Read the model definition and answer for the solid it produces. Units are mm, in the model's axes. A direction names the side the tool comes from. Give positions to 0.01 mm unless a question says otherwise; leave off trailing zeros. Loops run counter-clockwise (first coordinate to the right, second up) from the corner with the lowest first, then second, coordinate; pieces in that order, holes last.
(1) Find section B-B, the plane y = 0. Write down the section's boundary in (x, z), then the cut area to 3 significant figures.
(2) Determine the mould class of faces 6 (the face through (112, 7, 16)), 7 (the face through (7.048, 7.583, -12.942)), 8 (the face through (63.674, -12.447, -2.764)) for opening direction Z: pulls with the +Z half, pulls with the -Z half, needs draft (parallel to the pull), parting line crosses it, or undercut.
(3) Find section A-A, the plane z = 0. Write down the section's boundary in (x, y), then the cut area to 3 significant figures.
(4) Straight lines are drawn through the part: probe 1 along Y at (x, z) = (76, 0); probe 2 along Y at (x, z) = (72, -6); probe 3 along X at (y, z) = (-11, 14). For each, find the intervals that lie inside material, in ascending order.
(5) Find section C-C, the plane x = 90. Write down the section's boundary in (y, z).
(6) Each of these flat-tipped pins is pushed along its axis until it touches: P1, Ø5, axis at x = 94, z = 8.5, coming from the -Y side; P2, Ø8, axis at x = 59.5, y = -13, coming from the +Z side; P3, Ø0.8, axis at y = 15.5, z = 2, coming from the -X side. Where does it stop, or does it pass through?
(7) Which of the six approach directions +Z, -Z, +X, -X, +Y, -Y give full straight-line access (tool end or side, diameter ignored) to faces 1 (the face through (7, 15, 0)), 2 (the face through (7.048, -7.417, -13.038)), 3 (the face through (7, -15, 0)), 4 (the face through (14, 8, -14)), 5 (the face through (119.676, -4.956, 15.738))?
```python
from build123d import *

# Parameters (mm, degrees)
SKETCH1_R          = 18
EXTRUDE1_DEPTH     = 132
SKETCH2_R          = 12.75
CUT_EXTRUDE1_DEPTH = 135.432139014
SKETCH3_R          = 18
SKETCH3_R_2        = 16.5
CUT_EXTRUDE2_DEPTH = 15
CUT_EXTRUDE3_START = -20
SKETCH4_R          = 18
SKETCH4_R_2        = 16.5
CUT_EXTRUDE3_DEPTH = 20
FILLET1_R          = 0.5
SKETCH6_R          = 25
CUT_EXTRUDE4_DEPTH = 14


with BuildPart() as part:
    # Sketch1 → Extrude1 (new body)
    with BuildSketch(Plane(origin=(0, 0, 0), x_dir=(0, 0, -1), z_dir=(1, 0, 0))):
        Circle(SKETCH1_R)
    extrude(amount=EXTRUDE1_DEPTH)

    # Sketch2 → Cut-Extrude1 (cut, through all)
    with BuildSketch(Plane.ZY):
        Circle(SKETCH2_R)
    extrude(amount=-CUT_EXTRUDE1_DEPTH, mode=Mode.SUBTRACT)

    # Sketch3 → Cut-Extrude2 (cut)
    with BuildSketch(Plane.ZY):
        Circle(SKETCH3_R)
        Circle(SKETCH3_R_2, mode=Mode.SUBTRACT)
    extrude(amount=-CUT_EXTRUDE2_DEPTH, mode=Mode.SUBTRACT)

    # Sketch4 → Cut-Extrude3 (cut)
    with BuildSketch(Plane(origin=(132, 0, 0), x_dir=(0, 0, -1), z_dir=(1, 0, 0)).offset(CUT_EXTRUDE3_START)):
        with Locations(Location((0, 0, 0), (0, 0, 180))):
            Circle(SKETCH4_R)
        with Locations(Location((0, 0, 0), (0, 0, 180))):
            Circle(SKETCH4_R_2, mode=Mode.SUBTRACT)
    extrude(amount=CUT_EXTRUDE3_DEPTH, mode=Mode.SUBTRACT)

    # Fillet1
    fillet1_edges = [part.edges().sort_by_distance(p)[0] for p in [
        (15, 0, -16.5),
        (112, 0, -16.5),
    ]]
    fillet(fillet1_edges, radius=FILLET1_R)

    # Sketch5 → Cut-Revolve1 (revolve, cut)
    with BuildSketch(Plane.XY, mode=Mode.PRIVATE) as cut_revolve1_sk:
        with BuildLine():
            Line((119.041447752, -42.253356684), (137.021599533, -42.253356684))
            Line((137.021599533, -42.253356684), (137.021599533, 0))
            Line((137.021599533, 0), (132, 0))
            ThreePointArc((132, 0), (128.56354111, -13.941961258), (119.041447752, -24.689857401))
            Line((119.041447752, -24.689857401), (119.041447752, -42.253356684))
        make_face()
    revolve(cut_revolve1_sk.sketch.rotate(Axis((132, 0, 0), (-1, 0, 0)), 180), axis=Axis((132, 0, 0), (-1, 0, 0)), mode=Mode.SUBTRACT)

    # Sketch6 → Cut-Extrude4 (cut)
    with BuildSketch(Plane.ZY):
        Circle(SKETCH6_R)
        Polygon((-8.660254038, -15), (8.660254038, -15), (17.320508076, 0), (8.660254038, 15), (-8.660254038, 15), (-17.320508076, 0), align=None, mode=Mode.SUBTRACT)
    extrude(amount=-CUT_EXTRUDE4_DEPTH, mode=Mode.SUBTRACT)

    # Sketch7 → Cut-Revolve2 (revolve, cut)
    with BuildSketch(Plane.XY, mode=Mode.PRIVATE) as cut_revolve2_sk:
        Polygon((0, -14.5), (0, -24.5), (5.773502692, -24.5), align=None)
    revolve(cut_revolve2_sk.sketch.rotate(Axis((15, 0, 0), (-1, 0, 0)), 270), axis=Axis((15, 0, 0), (-1, 0, 0)), mode=Mode.SUBTRACT)


solid = part.part
```
Entries:
1. outline: (0, -14.5) - (1.15, -16.5) - (14.5, -16.5) arc R0.5 cw to (15, -17) - (15, -18) - (112, -18) - (112, -17) arc R0.5 cw to (112.5, -16.5) - (127.05, -16.5) arc R30 ccw to (129.16, -12.75) - (0, -12.75) - close; (0, 12.75) - (129.16, 12.75) arc R30 ccw to (127.05, 16.5) - (112.5, 16.5) arc R0.5 cw to (112, 17) - (112, 18) - (15, 18) - (15, 17) arc R0.5 cw to (14.5, 16.5) - (1.15, 16.5) - (0, 14.5) - close
1. area: 1,250 mm2
2. face 6: needs draft
2. face 7: pulls with the -Z half
2. face 8: undercut
3. outline: (0, -14.5) - (0.29, -15) - (14, -15) - (14, -16.5) - (14.5, -16.5) arc R0.5 cw to (15, -17) - (15, -18) - (112, -18) - (112, -17) arc R0.5 cw to (112.5, -16.5) - (127.05, -16.5) arc R30 ccw to (129.16, -12.75) - (0, -12.75) - close; (0, 12.75) - (129.16, 12.75) arc R30 ccw to (127.05, 16.5) - (112.5, 16.5) arc R0.5 cw to (112, 17) - (112, 18) - (15, 18) - (15, 17) arc R0.5 cw to (14.5, 16.5) - (14, 16.5) - (14, 15) - (0.29, 15) - (0, 14.5) - close
3. area: 1,210 mm2
4. probe 1: y = -18 to -12.75, 12.75 to 18
4. probe 2: y = -16.97 to -11.25, 11.25 to 16.97
4. probe 3: x = 15 to 112
5. outline: circle Ø36 at (0, 0); hole circle Ø25.5 at (0, 0)
6. P1: stops at y = -16.97
6. P2: stops at z = 15.59
6. P3: stops at x = 14
7. face 1: +Z, -Z, -X, +Y
7. face 2: -Z, -X, -Y
7. face 3: +Z, -Z, -X, -Y
7. face 4: -Z, -X, +Y
7. face 5: +X
